Here's the drawing with two shaded views (mm, measured from the low corner). I have some questions. Round coordinates to 2 decimals unless told otherwise and drop trailing zeros. Loops run counter-clockwise (first coordinate to the right, second up) from the corner with the lowest first, then second, coordinate; pieces in that order, holes last.
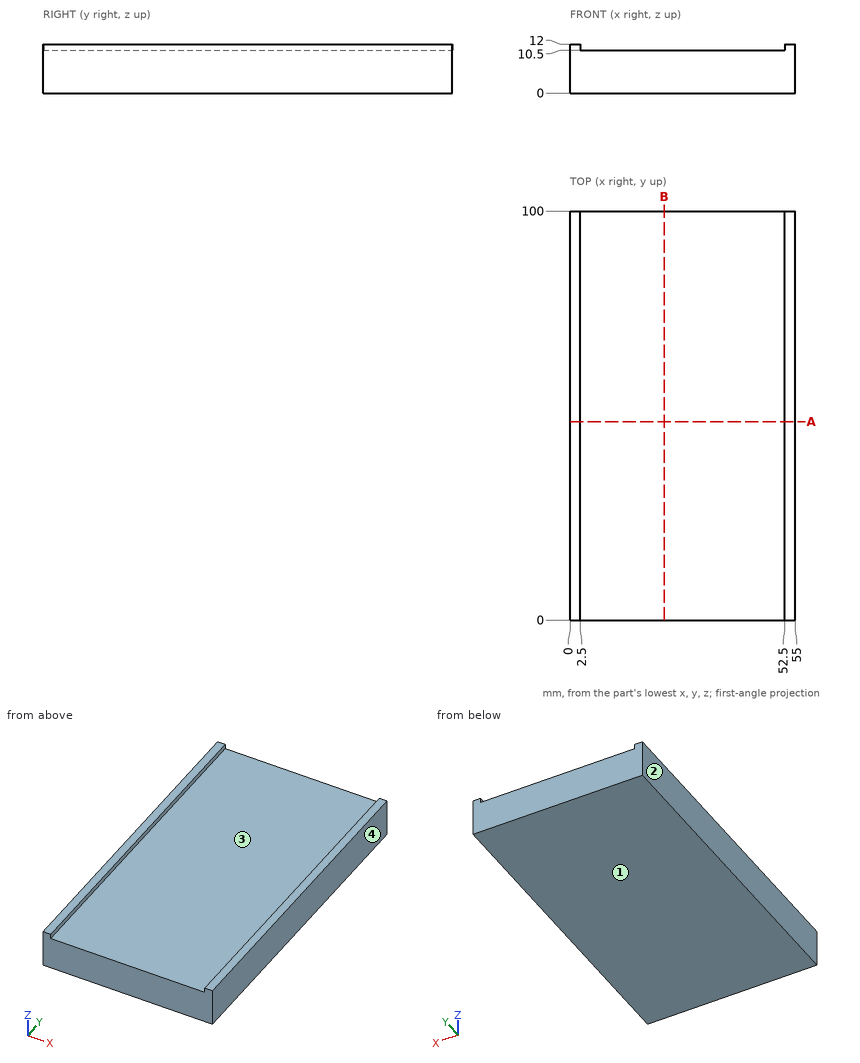
Item 1: If I drill on line 1 along Z through (x, y) = (21, 44), over which ranges is the centre line in solid material (lowest first)?
Results list:
line 1: z = 0 to 10.5
Item 2: If we section it at A-A, the plane y = 48.5: Please give me the cut outline in (x, z), then the cut area to 3 significant figures.
Results list:
outline: (0, 0) - (55, 0) - (55, 12) - (52.5, 12) - (52.5, 10.5) - (2.5, 10.5) - (2.5, 12) - (0, 12) - close
area: 585 mm2
Item 3: Will these pins go through, and if not, where does the flat tip stop? pin 1 (2 mm diameter, centred on x = 25, z = 7.5, fed in from -Y); pin 2 (3 mm diameter, centred on x = 25, y = 73, fed in from +Z).
Results list:
pin 1: stops at y = 0
pin 2: stops at z = 10.5
Item 4: If we section it at B-B, the plane x = 23: Please give me the cut outline in (y, z).
Results list:
outline: (0, 0) - (100, 0) - (100, 10.5) - (0, 10.5) - close
Item 5: We'd pull the mould along X, two halves only. Please class the marked faces 1, 2, 3 and 4: released by +X, released by -X, zero draft, split by the parting line, or undercut.
Results list:
face 1: zero draft
face 2: released by -X
face 3: undercut
face 4: released by +X
